Drawing for the job (mm, zero at the part's lowest x, y, z). Coordinates: 2 decimals unless noted, no trailing zeros. Order: outer loops, then holes, each group sorted by start corner. A loop starts at its lowest first (then second) coordinate and runs counter-clockwise, first axis right, second up. Notation, with made-up numbers: (16, 41.5) -> (71, 41.5) arc R14 ccw to (71, 60.5) -> close; hole circle Ø8 at (10, 0.5). An arc over 180 degrees is marked (long way). Write each question's results on one line, items separated by ' | '.
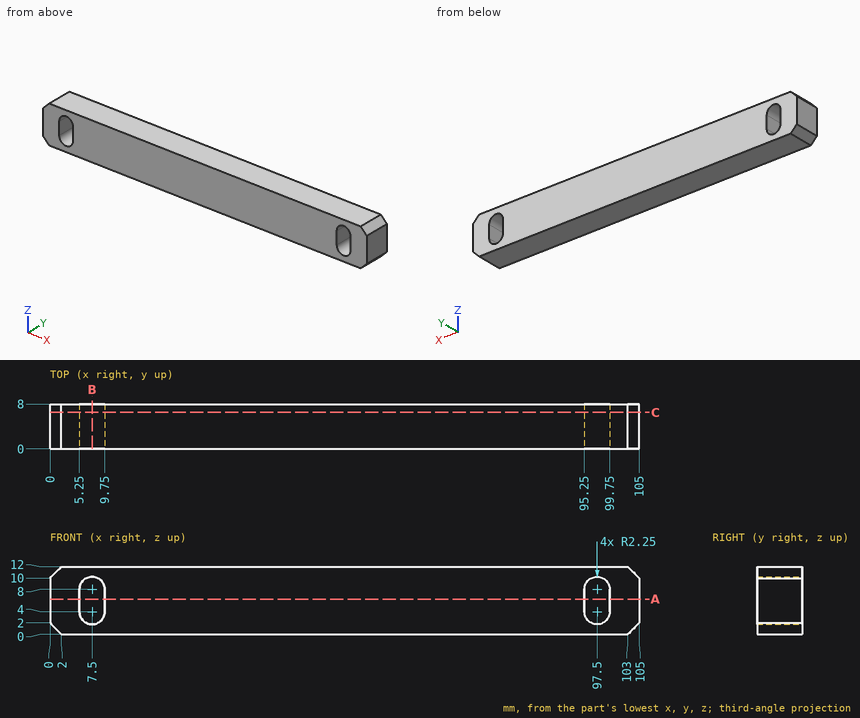
Item 1: Drill centre lines: line 1 (X direction, y = 6, z = 4.25); line 2 (X direction, y = 0.5, z = 2); line 3 (Z direction, x = 8.5, y = 6.75). Where is each one in solid material? Low to high. Write a range as from..to.
Answer:
line 1: x = 0..5.25, 9.75..95.25, 99.75..105 | line 2: x = 0..6.47, 8.53..96.47, 98.53..105 | line 3: z = 0..1.98, 10.02..12
Item 2: Slice it at C-C, the plane y = 6.5. List the corners of the cut face in (x, z).
Answer:
outline: (0, 2) -> (2, 0) -> (103, 0) -> (105, 2) -> (105, 10) -> (103, 12) -> (2, 12) -> (0, 10) -> close; hole (5.25, 4) arc R2.25 ccw to (9.75, 4) -> (9.75, 8) arc R2.25 ccw to (5.25, 8) -> close; hole (95.25, 4) arc R2.25 ccw to (99.75, 4) -> (99.75, 8) arc R2.25 ccw to (95.25, 8) -> close
Item 3: Slice it at B-B, the plane x = 7.5. List the corners of the cut face in (y, z), and give its area (3 significant figures).
Answer:
outline: (0, 0) -> (8, 0) -> (8, 1.75) -> (0, 1.75) -> close; (0, 10.25) -> (8, 10.25) -> (8, 12) -> (0, 12) -> close | area: 28.0 mm^2
Item 4: Slice it at A-A, the plane z = 6.25. List the corners of the cut face in (x, y).
Answer:
outline: (0, 0) -> (5.25, 0) -> (5.25, 8) -> (0, 8) -> close; (9.75, 0) -> (95.25, 0) -> (95.25, 8) -> (9.75, 8) -> close; (99.75, 0) -> (105, 0) -> (105, 8) -> (99.75, 8) -> close
